For this review, use the dimensioned drawing (mm, ordinates from the lowest corner) and the shaded views. Round coordinates to 2 decimals unless told otherwise and drop trailing zeros. Write each loop counter-clockwise with the first axis right and the second up, starting at its lowest first coordinate (ties: lowest second). Pieces come first, ordered by that corner, then holes. Notation, with made-up numbers: M 30.5,39 L 60.5,39 A30 ccw 60.5,66 Z; hole C 24,17 d8. An arc over 180 degrees is marked long. Use CSV: the item, a comma, the result in double quotes.
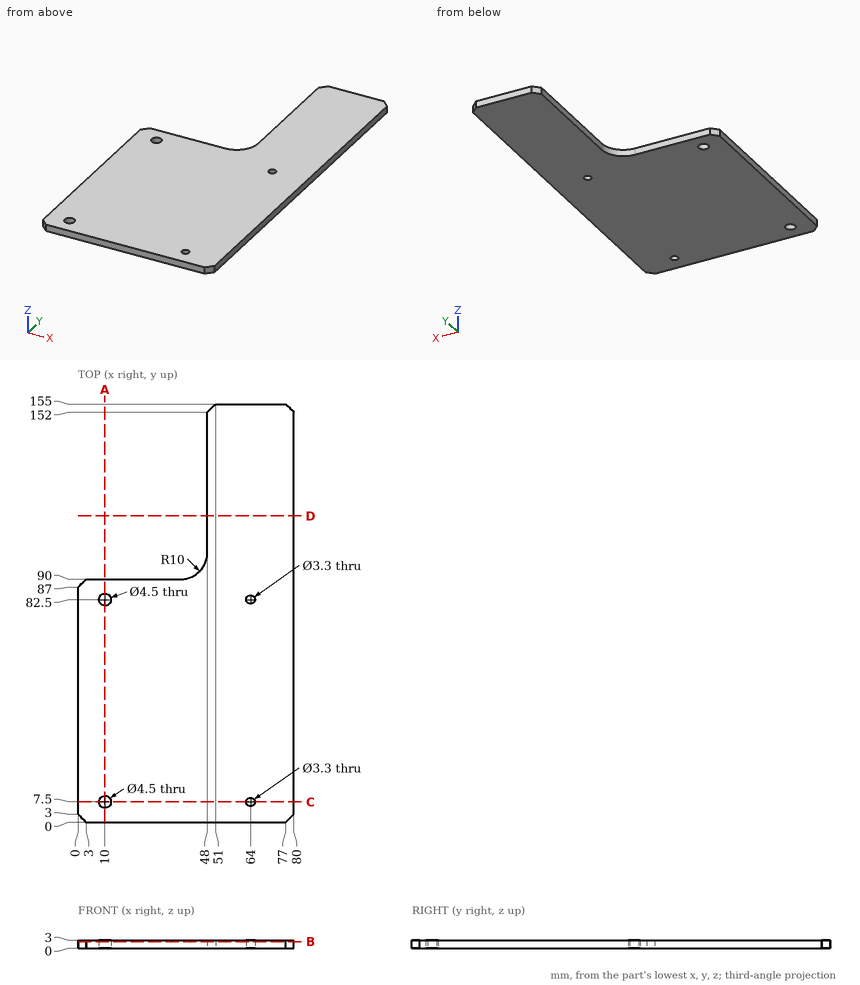
1) Add section D-D on y = 113.5. Write out the cut boundary in (x, z), then the cut area to 3 significant figures.
Answers:
outline,"M 48,0 L 80,0 L 80,3 L 48,3 Z"
area,"96.0 mm²"
2) For pin 1 Ø1.5 at (y, z) = (123, 1.5) entering from -X; pin 2 Ø4 at (x, y) = (64, 7.5) entering from +Z; pin 3 Ø4 at (x, y) = (10, 7.5) entering from +Z, all flat-tipped, find the tip position at first contact; note any pin that passes through.
Answers:
pin 1,"x = 48"
pin 2,"z = 3"
pin 3,"through"
3) Wall thickness on line 1 along Y through (x, z) = (10, 0.95); line 2 along Y through (x, z) = (64, 0.9); line 3 along Y through (x, z) = (34.5, 1.55): over which ranges is each line inside the solid? List them lowest first. Write a range as [from, to].
Answers:
line 1,"[0, 5.25], [9.75, 80.25], [84.75, 90]"
line 2,"[0, 5.85], [9.15, 80.85], [84.15, 155]"
line 3,"[0, 90]"
4) Add section C-C on y = 7.5. Write out the cut boundary in (x, z).
Answers:
outline,"M 0,0 L 7.75,0 L 7.75,3 L 0,3 Z; M 12.25,0 L 62.35,0 L 62.35,3 L 12.25,3 Z; M 65.65,0 L 80,0 L 80,3 L 65.65,3 Z"
5) Add section A-A on x = 10. Write out the cut boundary in (y, z).
Answers:
outline,"M 0,0 L 5.25,0 L 5.25,3 L 0,3 Z; M 9.75,0 L 80.25,0 L 80.25,3 L 9.75,3 Z; M 84.75,0 L 90,0 L 90,3 L 84.75,3 Z"
6) Add section B-B on z = 2.5. Write out the cut boundary in (x, y).
Answers:
outline,"M 0,3 L 3,0 L 77,0 L 80,3 L 80,152 L 77,155 L 51,155 L 48,152 L 48,100 A10 cw 38,90 L 3,90 L 0,87 Z; hole C 10,7.5 d4.5; hole C 10,82.5 d4.5; hole C 64,7.5 d3.3; hole C 64,82.5 d3.3"
